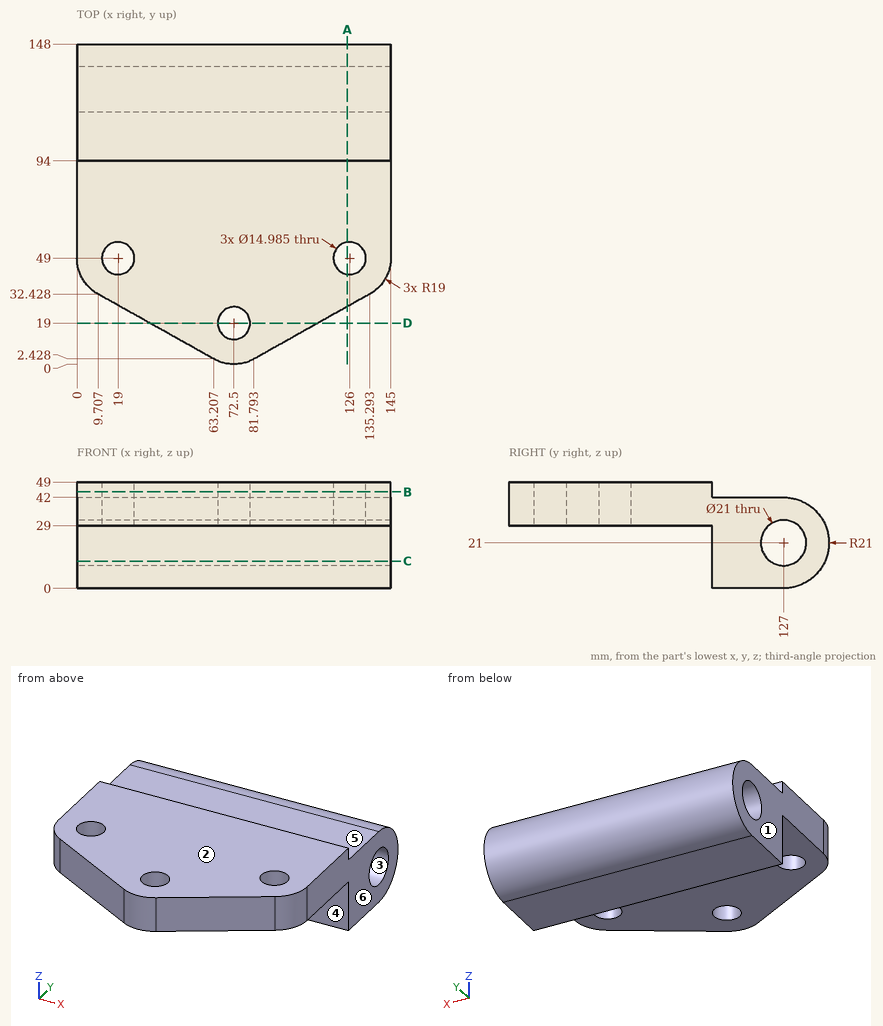
For this review, use the dimensioned drawing (mm, ordinates from the lowest corner) and the shaded views. A direction names the side the tool comes from. Round coordinates to 2 decimals unless told otherwise and drop trailing zeros. Write each loop counter-clockwise with the first axis right and the second up, starting at its lowest first coordinate (ties: lowest second). Pieces come first, ordered by that corner, then holes. Notation, with made-up numbers: M 34,-26.75 L 52,-26.75 A22 cw 52,-14.75 Z; hole C 24,15 d8. An arc over 180 degrees is marked long. Answer as CSV lines item,"result". Start each with the question number.
Q1. Consider section D-D, the plane y = 19. Give the boundary of the cut face in (x, z).
Q2. Clearance check with flat-ended pins moving along their axes: P1, Ø19.5, axis at x = 72.5, y = 19, coming from the +Z side; P2, Ø4, axis at x = 52.5, z = 8.5, coming from the +Y side; P3, Ø23, axis at x = 77, z = 21, coming from the -Y side; P4, Ø16.5, axis at x = 66, y = 111.5, coming from the +Z side. State where each tip first meets the part, or that it passes through.
Q3. Consider section A-A, the plane x = 125. Give the boundary of the cut face in (y, z) (1 decimal).
Q4. Consider section B-B, the plane z = 44.5. Give the boundary of the cut face in (x, y) (1 decimal), then the cut area to 3 significant figures.
Q5. Wall thickness on line 1 along Z through (x, y) = (47.5, 79.5); line 2 along Y through (x, z) = (126, 43.5) (1 decimal); line 3 along Y through (x, z) = (68, 24.5) (1 decimal): over which ranges is each line inside the solid? List them lowest first.
Q6. Consider section C-C, the plane z = 12.5. Give the boundary of the cut face in (x, y) (1 decimal), then the cut area to 3 significant figures.
Q7. Tool access review of the marked faces 4, 5 and 6: name each direction out of +Z, -Z, +X, -X, +Y, -Y from which nothing blocks a thin tool from reaching the whole face with its end or side.
Q8. The part is to be moulded in two halves that separate along Z. For the marked faces 1, 2 and 3, say which applies: +Z half, -Z half, draft (parallel to the pull), parting line (faces both ways), or undercut.
Result set:
1,outline,"M 33.65,29 L 65.01,29 L 65.01,49 L 33.65,49 Z; M 79.99,29 L 111.35,29 L 111.35,49 L 79.99,49 Z"
2,P1,"stops at z = 49"
2,P2,"stops at y = 145.19"
2,P3,"stops at y = 0"
2,P4,"stops at z = 42"
3,outline,"M 26.7,29 L 41.6,29 L 41.6,49 L 26.7,49 Z; M 56.4,29 L 94,29 L 94,0 L 127,0 A21 ccw 127,42 L 94,42 L 94,49 L 56.4,49 Z; hole C 127,21 d21"
4,outline,"M 0,49 A19 ccw 9.7,32.4 L 63.2,2.4 A19 ccw 81.8,2.4 L 135.3,32.4 A19 ccw 145,49 L 145,94 L 0,94 Z; hole C 19,49 d15; hole C 72.5,19 d15; hole C 126,49 d15"
4,area,"10,500 mm²"
5,line 1,"z = 29 to 49"
5,line 2,"y = 27.2 to 41.5, 56.5 to 94"
5,line 3,"y = 94 to 117.1, 136.9 to 147.7"
6,outline,"M 0,94 L 145,94 L 145,120.8 L 0,120.8 Z; M 0,133.2 L 145,133.2 L 145,146.2 L 0,146.2 Z"
6,area,"5,780 mm²"
7,face 4,"-Z, +X, -X, -Y"
7,face 5,"+Z, +X, -X, +Y"
7,face 6,"+Z, -Z, +X, +Y, -Y"
8,face 1,"draft"
8,face 2,"+Z half"
8,face 3,"undercut"
